For this review, take the finished solid that the model builds, in its own axes (mm). A direction names the side the tool comes from. Round coordinates to 2 decimals unless told otherwise and drop trailing zeros. Order: outer loops, then holes, each group sorted by start corner. A loop starts at its lowest first (then second) coordinate and runs counter-clockwise, first axis right, second up. Notation, with made-up numbers: (7.25, 3.5) -> (61.25, 3.5) arc R12 ccw to (61.25, 8.5) -> close; hole circle Ø6 at (12.5, 7). An arc over 180 degrees is marked (long way). Put each result on its own line as item: value. Start each with the question number.
```python
from build123d import *

# Parameters (mm, degrees)
SKETCH1_R                              = 24.75
BOSS_EXTRUDE1_DEPTH                    = 9
CUT_EXTRUDE1_START                     = -7
CUT_EXTRUDE1_DEPTH                     = 44.140351409
SKETCH3_R                              = 2.75
CUT_EXTRUDE2_DEPTH                     = 7
CIRPATTERN1_COUNT                      = 3
SKETCH5_R                              = 4
BOSS_EXTRUDE2_DEPTH                    = 1
SKETCH6_R                              = 3.5
BOSS_EXTRUDE3_DEPTH                    = 3
F_5_0MM_BLIND_DOWEL_HOLE_1_D           = 5
F_5_0MM_BLIND_DOWEL_HOLE_1_DEPTH       = 5
F_5_0MM_BLIND_DOWEL_HOLE_1_CSINK_D     = 5.05
F_5_0MM_BLIND_DOWEL_HOLE_1_CSINK_ANGLE = 90
F_5_0MM_BLIND_DOWEL_HOLE_1_TIP         = 1.502151548
CUT_EXTRUDE3_START                     = 7
CUT_EXTRUDE3_DEPTH                     = 5
SKETCH9_R                              = 8
CUT_EXTRUDE4_DEPTH                     = 5


with BuildPart() as part:
    # Sketch1 → Boss-Extrude1 (new body)
    with BuildSketch(Plane(origin=(0, 0, 0), x_dir=(1, 0, 0), z_dir=(0, 1, 0))):
        with Locations(Location((0, 0, 0), (0, 0, 270))):
            Circle(SKETCH1_R)
    extrude(amount=BOSS_EXTRUDE1_DEPTH)

    # Sketch2 → Cut-Extrude1 (cut)
    with BuildSketch(Plane(origin=(0, 9, 0), x_dir=(1, 0, 0), z_dir=(0, 1, 0)).offset(CUT_EXTRUDE1_START)):
        with BuildLine():
            Line((-4.25, 21.25), (-4.25, 27.920433859))
            Line((-4.25, 27.920433859), (4.25, 27.920433859))
            Line((4.25, 27.920433859), (4.25, 21.25))
            ThreePointArc((4.25, 21.25), (0, 17), (-4.25, 21.25))
        make_face()
    cut_extrude1 = extrude(amount=CUT_EXTRUDE1_DEPTH, mode=Mode.SUBTRACT)

    # Sketch3 → Cut-Extrude2 (cut)
    with BuildSketch(Plane(origin=(0, 2, 0), x_dir=(1, 0, 0), z_dir=(0, 1, 0))):
        with Locations(Location((0, 21.25, 0), (0, 0, 270))):
            Circle(SKETCH3_R)
    cut_extrude2 = extrude(amount=-CUT_EXTRUDE2_DEPTH, mode=Mode.SUBTRACT)

    # CirPattern1: Cut-Extrude1, Cut-Extrude2 ×3 about axis
    cirpattern1_axis = Axis((0, 0, 0), (0, 1, 0))
    add([cut_extrude1.rotate(cirpattern1_axis, i * 360 / CIRPATTERN1_COUNT) for i in range(1, CIRPATTERN1_COUNT)], mode=Mode.SUBTRACT)
    add([cut_extrude2.rotate(cirpattern1_axis, i * 360 / CIRPATTERN1_COUNT) for i in range(1, CIRPATTERN1_COUNT)], mode=Mode.SUBTRACT)

    # Sketch5 → Boss-Extrude2 (add)
    with BuildSketch(Plane(origin=(0, 9, 0), x_dir=(1, 0, 0), z_dir=(0, 1, 0))):
        with Locations(Location((0, -12.75, 0), (0, 0, 270))):
            Circle(SKETCH5_R)
    extrude(amount=BOSS_EXTRUDE2_DEPTH)

    # Sketch6 → Boss-Extrude3 (add)
    with BuildSketch(Plane(origin=(0, 9, 0), x_dir=(1, 0, 0), z_dir=(0, 1, 0))):
        with Locations(Location((0, -12.75, 0), (0, 0, 270))):
            Circle(SKETCH6_R)
    extrude(amount=BOSS_EXTRUDE3_DEPTH)

    # Ø5.0mm blind dowel hole 1
    with Locations(Plane(origin=(0, 12, 0), x_dir=(1, 0, 0), z_dir=(0, 1, 0))):
        with Locations((0, -12.75)):
            CounterSinkHole(F_5_0MM_BLIND_DOWEL_HOLE_1_D / 2, F_5_0MM_BLIND_DOWEL_HOLE_1_CSINK_D / 2, depth=F_5_0MM_BLIND_DOWEL_HOLE_1_DEPTH, counter_sink_angle=F_5_0MM_BLIND_DOWEL_HOLE_1_CSINK_ANGLE)
            with Locations((0, 0, -(F_5_0MM_BLIND_DOWEL_HOLE_1_DEPTH + F_5_0MM_BLIND_DOWEL_HOLE_1_TIP / 2))):  # 118° drill point
                Cone(0, F_5_0MM_BLIND_DOWEL_HOLE_1_D / 2, F_5_0MM_BLIND_DOWEL_HOLE_1_TIP, mode=Mode.SUBTRACT)

    # Sketch4 → Cut-Extrude3 (cut)
    with BuildSketch(Plane(origin=(0, 2, 0), x_dir=(1, 0, 0), z_dir=(0, 1, 0)).offset(CUT_EXTRUDE3_START)):
        with BuildLine():
            ThreePointArc((10.559685096, -12.678448276), (0, 16.5), (-10.559685096, -12.678448276))
            ThreePointArc((-10.559685096, -12.678448276), (-9.090434755, -13.132688982), (-7.733102721, -12.409722222))
            ThreePointArc((-7.733102721, -12.409722222), (0, -8.75), (7.733102721, -12.409722222))
            ThreePointArc((7.733102721, -12.409722222), (9.090434755, -13.132688982), (10.559685096, -12.678448276))
        make_face()
    extrude(amount=-CUT_EXTRUDE3_DEPTH, mode=Mode.SUBTRACT)

    # Sketch9 → Cut-Extrude4 (cut)
    with BuildSketch(Plane.XZ):
        with Locations(Location((0, 0, 0), (0, 0, 270))):
            Circle(SKETCH9_R)
    extrude(amount=-CUT_EXTRUDE4_DEPTH, mode=Mode.SUBTRACT)


solid = part.part
```
Item 1: Consider section A-A, the plane y = 2.75. Write out the cut boundary in (x, z) (3 decimals).
Item 2: Consider section B-B, the plane z = 0. Write out the cut boundary in (x, y).
Item 3: Consider section C-C, the plane z = -5. Write out the cut boundary in (x, y) (3 decimals), plus the area to 3 significant figures.
Item 4: Tool access review of faces 1 (the face through (17.65, 5.45, 15.1)), 2 (the face through (-4.25, 5, -23)), 3 (the face through (14.677, 5.451, 8.581)): name each direction out of +Z, -Z, +X, -X, +Y, -Y from which nothing blocks a thin tool from reaching the whole face with its end or side.
Item 5: Consider section D-D, the plane z = 11.5. Count the separate pieces of the cut face and the enclosed holes in it, plus the area to 3 significant figures.
Item 6: Insertion check: pin 1 Ø1.6 at (y, z) = (5.5, -22) entering from +X; pin 2 Ø10 at (x, z) = (-20, 11.5) entering from +Y; pin 3 Ø5 at (x, y) = (-3.5, 9.5) entering from +Z; pin 4 Ø4.5 at (x, z) = (18.4, 10.63) entering from -Y. Each pin has a flat end and moves straight along its axis. Give the tip position at first contact, or say it passes through.
Item 7: For L1, parallel to Z at x = 2, y = 1.5; L2, parallel to Z at x = 2, y = 7.25; L3, parallel to Y at x = 19, z = -6.5, list the stretches that pass through material, from the lowest coordinate up.
Evaluation:
1. outline: (-23.241, 8.511) arc R24.75 ccw to (-4.25, -24.382) -> (-4.25, -21.25) arc R4.25 cw to (4.25, -21.25) -> (4.25, -24.382) arc R24.75 ccw to (23.241, 8.511) -> (20.528, 6.944) arc R4.25 cw to (16.278, 14.306) -> (18.991, 15.872) arc R24.75 ccw to (-18.991, 15.872) -> (-16.278, 14.306) arc R4.25 cw to (-20.528, 6.944) -> close; hole circle Ø16 at (0, 0)
2. outline: (-24.75, 0) -> (-8, 0) -> (-8, 4) -> (-16.5, 4) -> (-16.5, 9) -> (-24.75, 9) -> close; (8, 0) -> (24.75, 0) -> (24.75, 9) -> (16.5, 9) -> (16.5, 4) -> (8, 4) -> close
3. outline: (-24.24, 0) -> (-6.245, 0) -> (-6.245, 4) -> (-15.724, 4) -> (-15.724, 9) -> (-24.24, 9) -> close; (6.245, 0) -> (24.24, 0) -> (24.24, 9) -> (15.724, 9) -> (15.724, 4) -> (6.245, 4) -> close
3. area: 229 mm^2
4. face 1: +X, +Y
4. face 2: -Z, +Y
4. face 3: +Y
5. separate pieces: 3
5. enclosed holes: 0
5. area: 214 mm^2
6. pin 1: stops at x = 12.77
6. pin 2: stops at y = 9
6. pin 3: stops at z = 24.73
6. pin 4: passes through
7. L1: z = -24.67 to -23.14, -19.36 to -7.75, 7.75 to 24.67
7. L2: z = -17.5 to -16.38, 8.95 to 11.25, 14.25 to 24.67
7. L3: y = 0 to 9
